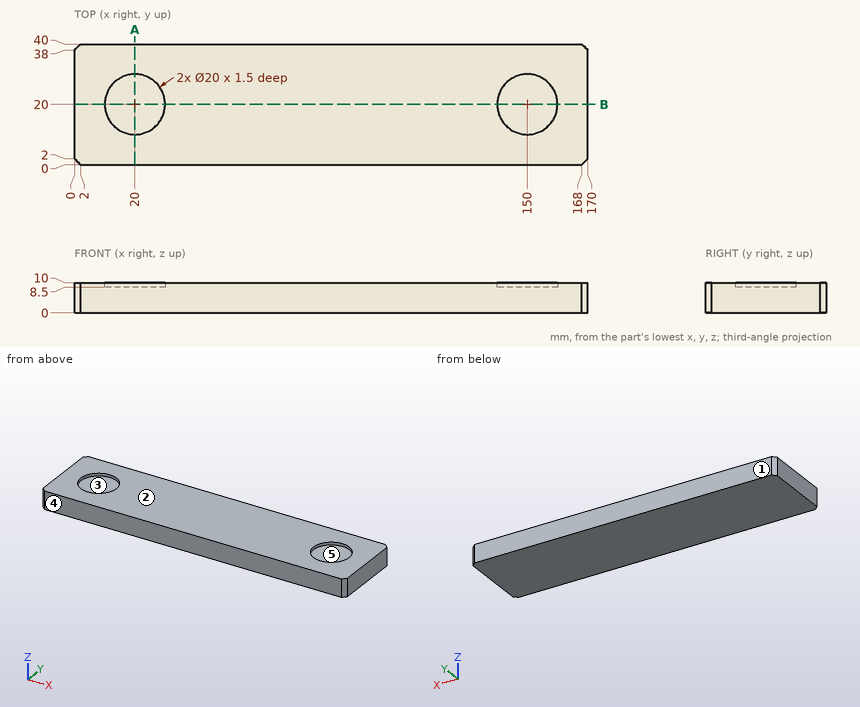
Answer from the drawing. Dimensions are ordinates in mm from the lowest x, y and z of the part. A direction names the side the tool comes from. Coordinates: 2 decimals unless noted, no trailing zeros. Write each loop counter-clockwise with the first axis right and the second up, starting at its lowest first coordinate (ties: lowest second). Pieces come first, ordered by that corner, then holes. Notation, with made-up numbers: M -14.5,19.5 L 9.5,19.5 A19 cw 9.5,32.5 Z; hole C 67,80 d6. An arc over 180 degrees is marked long. Put each result on its own line as item: value. Start each with the question number.
1. Which of the six approach directions +Z, -Z, +X, -X, +Y, -Y give full straight-line access (tool end or side, diameter ignored) to the marked faces 4 and 5?
2. For a pull along Y with two mould halves and no side action, classify the marked faces 1, 2 and 3 as pulls with the +Y half, pulls with the -Y half, needs draft (parallel to the pull), parting line crosses it, or undercut.
3. A cutting plane is placed at A-A on x = 20. Write down the section's boundary in (y, z), then the cut area to 3 significant figures.
4. A flat-ended cylindrical pin translates along its axis: P1, Ø18, axis at x = 150, y = 20, coming from the +Z side. Find the tip coordinate at first contact, or state that the pin passes through.
5. Consider line 1 (Y direction, x = 150, z = 9.25); line 2 (X direction, y = 27, z = 9). Determine where each line is inside the solid, lowest interval first. Write a range as from..to.
6. A cutting plane is placed at B-B on y = 20. Write down the section's boundary in (x, z), then the cut area to 3 significant figures.
Resolved:
1. face 4: +Z, -Z, +X, -X, -Y
1. face 5: +Z
2. face 1: pulls with the +Y half
2. face 2: needs draft
2. face 3: undercut
3. outline: M 0,0 L 40,0 L 40,10 L 30,10 L 30,8.5 L 10,8.5 L 10,10 L 0,10 Z
3. area: 370 mm2
4. P1: stops at z = 8.5
5. line 1: y = 0..10, 30..40
5. line 2: x = 0..12.86, 27.14..142.86, 157.14..170
6. outline: M 0,0 L 170,0 L 170,10 L 160,10 L 160,8.5 L 140,8.5 L 140,10 L 30,10 L 30,8.5 L 10,8.5 L 10,10 L 0,10 Z
6. area: 1,640 mm2
